Could you check a few things on this model? Use its own coordinates, in mm. A direction names the side the tool comes from. Round coordinates to 2 decimals unless told otherwise and drop trailing zeros. Loops run counter-clockwise (first coordinate to the right, second up) from the corner with the lowest first, then second, coordinate; pieces in that order, holes last.
from build123d import *

# Parameters (mm, degrees)
SKETCH_1_W               = 60
SKETCH_1_H               = 60
EXTRUDE_1_DEPTH          = 25
SKETCH_2_R               = 30
EXTRUDE_2_DEPTH          = 48
SKETCH_3_R               = 20
EXTRUDE_3_DEPTH          = 3
SKETCH_4_R               = 8.5
EXTRUDE_4_DEPTH          = 2
SKETCH_5_R               = 7
EXTRUDE_5_DEPTH          = 30
SKETCH_7_R               = 3.175
CUT_EXTRUDE_1_DEPTH      = 21
SKETCH_8_R               = 19
CUT_EXTRUDE_2_DEPTH      = 2
PATTERN_CIRCULAR_1_COUNT = 4
CHAMFER_1_SIZE           = 2
SKETCH_17_W              = 4
SKETCH_17_H              = 5
EXTRUDE_6_DEPTH          = 27.5
CHAMFER_2_SIZE           = 0.5


with BuildPart() as part:
    # 草图1 → 凸台-拉伸1 (new body)
    with BuildSketch(Plane.XY):
        Rectangle(SKETCH_1_W, SKETCH_1_H)
    extrude(amount=EXTRUDE_1_DEPTH)

    # 草图2 → 凸台-拉伸2 (add)
    with BuildSketch(Plane(origin=(0, 0, 0), x_dir=(-1, 0, 0), z_dir=(0, 0, -1))):
        Circle(SKETCH_2_R)
    extrude(amount=EXTRUDE_2_DEPTH)

    # 草图3 → 凸台-拉伸3 (add)
    with BuildSketch(Plane(origin=(0, 0, -48), x_dir=(-1, 0, 0), z_dir=(0, 0, -1))):
        Circle(SKETCH_3_R)
    extrude(amount=EXTRUDE_3_DEPTH)

    # 草图4 → 凸台-拉伸4 (add)
    with BuildSketch(Plane(origin=(0, 0, -51), x_dir=(-1, 0, 0), z_dir=(0, 0, -1))):
        Circle(SKETCH_4_R)
    extrude(amount=EXTRUDE_4_DEPTH)

    # 草图5 → 凸台-拉伸5 (add)
    with BuildSketch(Plane(origin=(0, 0, -53), x_dir=(-1, 0, 0), z_dir=(0, 0, -1))):
        Circle(SKETCH_5_R)
    extrude(amount=EXTRUDE_5_DEPTH)

    # 草图7 → 切除-拉伸1 (cut)
    with BuildSketch(Plane.XY.offset(25)):
        Circle(SKETCH_7_R)
    extrude(amount=-CUT_EXTRUDE_1_DEPTH, mode=Mode.SUBTRACT)

    # 草图8 → 切除-拉伸2 (cut)
    with BuildSketch(Plane.XY.offset(25)):
        Circle(SKETCH_8_R)
    extrude(amount=-CUT_EXTRUDE_2_DEPTH, mode=Mode.SUBTRACT)

    # 草图10 → M4 螺纹孔1 (revolve, cut)
    with BuildSketch(Plane(origin=(23.5, 23.5, 25), x_dir=(0, -1, 0), z_dir=(1, 0, 0))):
        Polygon((0, 0), (0, 12.491420021), (1.65, 11.5), (1.65, 0), align=None)
    hole_wizard_m4_1 = revolve(axis=Axis((23.5, 23.5, 31.35), (0, 0, -1)), mode=Mode.SUBTRACT)

    # 草图15 → M5 螺纹孔1 (revolve, cut)
    with BuildSketch(Plane(origin=(-18.384776311, 18.384776311, -48), x_dir=(0, 1, 0), z_dir=(1, 0, 0))):
        Polygon((0, 0), (0, 13.2618073), (2.1, 12), (2.1, 0), align=None)
    hole_wizard_m5_1 = revolve(axis=Axis((-18.384776311, 18.384776311, -54.35), (0, 0, 1)), mode=Mode.SUBTRACT)

    # 阵列(圆周)1: M4 螺纹孔1, M5 螺纹孔1 ×4 about axis
    pattern_circular_1_axis = Axis((0, 0, 0), (0, 0, 1))
    add([hole_wizard_m4_1.rotate(pattern_circular_1_axis, i * 360 / PATTERN_CIRCULAR_1_COUNT) for i in range(1, PATTERN_CIRCULAR_1_COUNT)], mode=Mode.SUBTRACT)
    add([hole_wizard_m5_1.rotate(pattern_circular_1_axis, i * 360 / PATTERN_CIRCULAR_1_COUNT) for i in range(1, PATTERN_CIRCULAR_1_COUNT)], mode=Mode.SUBTRACT)

    # 倒角1
    chamfer_1_edges = [part.edges().sort_by_distance(p)[0] for p in [
        (30, -30, 12.5),
        (-30, -30, 12.5),
        (-30, 30, 12.5),
        (30, 30, 12.5),
    ]]
    chamfer(chamfer_1_edges, length=CHAMFER_1_SIZE)

    # 草图17 → 凸台-拉伸6 (add)
    with BuildSketch(Plane(origin=(0, 0, -83), x_dir=(-1, 0, 0), z_dir=(0, 0, -1))):
        with Locations((7, 0)):
            Rectangle(SKETCH_17_W, SKETCH_17_H)
    extrude(amount=-EXTRUDE_6_DEPTH)

    # 倒角2
    chamfer_2_edges = [part.edges().sort_by_distance(p)[0] for p in [
        (30, 0, -48),
        (7, 0, -83),
    ]]
    chamfer(chamfer_2_edges, length=CHAMFER_2_SIZE)


solid = part.part
Item 1: If we section it at A-A, the plane z = -40: Please give me the cut outline in (x, y).
Results list:
outline: circle Ø60 at (0, 0); hole circle Ø4.2 at (-18.38, -18.38); hole circle Ø4.2 at (-18.38, 18.38); hole circle Ø4.2 at (18.38, -18.38); hole circle Ø4.2 at (18.38, 18.38)
Item 2: If we section it at B-B, the plane z = -72: Please give me the cut outline in (x, y), then the cut area to 3 significant figures.
Results list:
outline: (-9, -2.5) - (-6.54, -2.5) arc R7 ccw (long way) to (-6.54, 2.5) - (-9, 2.5) - close
area: 165 mm2
Item 3: We'd pull the mould along Y, two halves only. Please class faces 4 (the conical face through (18.581, 18.692, -34.957)), 5 (the flat face through (0, -9, -51)), 6 (the conical face through (6.637, 0.258, -82.858)): released by +Y, released by -Y, zero draft, split by the parting line, or undercut.
Results list:
face 4: undercut
face 5: zero draft
face 6: split by the parting line
Item 4: Will these pins go through, and if not, where does the flat tip stop? pin 1 (2 mm diameter, centred on x = -4.5, z = -68, fed in from +Y); pin 2 (2.5 mm diameter, centred on x = -7, z = -69.5, fed in from +Y); pin 3 (3 mm diameter, centred on x = -13.5, z = -14.5, fed in from -Y).
Results list:
pin 1: stops at y = 6.06
pin 2: stops at y = 3.99
pin 3: stops at y = -27.5
Item 5: For faces 1 (the cylindrical face through (4.336, -19.524, -49.479)), 2 (the flat face through (-8, 2.5, -69)), 3 (the flat face through (0, -4, 23)), which set-ups out of +Z, -Z, +X, -X, +Y, -Y let a thin tool reach every point of the face, with its end or its side?
Results list:
face 1: -Z
face 2: -Z, -X, +Y
face 3: +Z
Item 6: If I drill on line 1 along Z through (x, y) = (-8.5, 1); line 2 along Y through (x, z) = (0, 24); line 3 along Z through (x, y) = (-28, -6), over which ranges is the centre line in solid material (lowest first)?
Results list:
line 1: z = -83 to -55.5, -51 to 23
line 2: y = -30 to -19, 19 to 30
line 3: z = -48 to 25
Item 7: If we section it at C-C, the plane z = -20: Please give me the cut outline in (x, y), then the cut area to 3 significant figures.
Results list:
outline: circle Ø60 at (0, 0)
area: 2,830 mm2
